```python
from build123d import *

# Parameters (mm, degrees)
WEB_1_DEPTH                   = 22
CRANKPIN_1_SKETCH_R           = 22.5
CRANKPIN_1_45_DEPTH           = 35
WEB_2_DEPTH                   = 25
CRANKPIN_2_SKETCH_R           = 22.5
CRANKPIN_2_45_DEPTH           = 35
WEB_3_DEPTH                   = 22
CENTRE_MAIN_JOURNAL_SKETCH_R  = 25
CENTRE_MAIN_JOURNAL_50_DEPTH  = 45
WEB_4_DEPTH                   = 22
CRANKPIN_3_SKETCH_R           = 22.5
CRANKPIN_3_45_DEPTH           = 35
WEB_5_DEPTH                   = 25
CRANKPIN_4_SKETCH_R           = 22.5
CRANKPIN_4_45_DEPTH           = 35
WEB_6_DEPTH                   = 22
FRONT_START                   = 45
FRONT_JOURNAL_SKETCH_R        = 22.5
FRONT_JOURNAL_45_DEPTH        = 45
FRONT_SHAFT_SKETCH_R          = 25
FRONT_SHAFT_50_DEPTH          = 100
NOSE_SKETCH_R                 = 12.5
NOSE_25_DEPTH                 = 20
FLANGE_BOLT_HOLES_SKETCH_R    = 6
FLANGE_BOLT_HOLES_4X_12_DEPTH = 20
KEYWAY_SKETCH_W               = 5
KEYWAY_SKETCH_H               = 10
KEYWAY_10X5_DEPTH             = 110


with BuildPart() as part:
    # Flange Profile Sketch → Flange and Rear Shaft (revolve)
    with BuildSketch(Plane.XY, mode=Mode.PRIVATE) as flange_and_rear_shaft_sk:
        Polygon((0, 0), (0, 60), (16, 60), (16, 22.5), (78, 22.5), (78, 0), align=None)
    revolve(flange_and_rear_shaft_sk.sketch.rotate(Axis((-89.086419753, 0, 0), (1, 0, 0)), 90), axis=Axis((-89.086419753, 0, 0), (1, 0, 0)))

    # Web 1 Sketch → Web 1 (add)
    with BuildSketch(Plane(origin=(78, 0, 0), x_dir=(0, 0, -1), z_dir=(1, 0, 0))):
        with BuildLine():
            Line((0, -27.5), (-40, -27.5))
            ThreePointArc((-40, -27.5), (-67.5, 0), (-40, 27.5))
            Line((-40, 27.5), (0, 27.5))
            ThreePointArc((0, 27.5), (27.5, 0), (0, -27.5))
        make_face()
    extrude(amount=WEB_1_DEPTH)

    # Crankpin 1 Sketch → Crankpin 1 Ø45 (add)
    with BuildSketch(Plane(origin=(100, 0, 0), x_dir=(0, 0, -1), z_dir=(1, 0, 0))):
        with Locations((-40, 0)):
            Circle(CRANKPIN_1_SKETCH_R)
    extrude(amount=CRANKPIN_1_45_DEPTH)

    # Web 2 Sketch → Web 2 (add)
    with BuildSketch(Plane(origin=(135, 0, 0), x_dir=(0, 0, -1), z_dir=(1, 0, 0))):
        with BuildLine():
            Line((-40, 27.5), (40, 27.5))
            ThreePointArc((40, 27.5), (67.5, 0), (40, -27.5))
            Line((40, -27.5), (-40, -27.5))
            ThreePointArc((-40, -27.5), (-67.5, 0), (-40, 27.5))
        make_face()
    extrude(amount=WEB_2_DEPTH)

    # Crankpin 2 Sketch → Crankpin 2 Ø45 (add)
    with BuildSketch(Plane(origin=(160, 0, 0), x_dir=(0, 0, -1), z_dir=(1, 0, 0))):
        with Locations((40, 0)):
            Circle(CRANKPIN_2_SKETCH_R)
    extrude(amount=CRANKPIN_2_45_DEPTH)

    # Web 3 Sketch → Web 3 (add)
    with BuildSketch(Plane(origin=(195, 0, 0), x_dir=(0, 0, -1), z_dir=(1, 0, 0))):
        with BuildLine():
            Line((40, -27.5), (0, -27.5))
            ThreePointArc((0, -27.5), (-27.5, 0), (0, 27.5))
            Line((0, 27.5), (40, 27.5))
            ThreePointArc((40, 27.5), (67.5, 0), (40, -27.5))
        make_face()
    extrude(amount=WEB_3_DEPTH)

    # Centre Main Journal Sketch → Centre Main Journal Ø50 (add)
    with BuildSketch(Plane(origin=(217, 0, 0), x_dir=(0, 0, -1), z_dir=(1, 0, 0))):
        with Locations(Location((0, 0, 0), (0, 0, 180))):
            Circle(CENTRE_MAIN_JOURNAL_SKETCH_R)
    extrude(amount=CENTRE_MAIN_JOURNAL_50_DEPTH)

    # Web 4 Sketch → Web 4 (add)
    with BuildSketch(Plane(origin=(262, 0, 0), x_dir=(0, 0, -1), z_dir=(1, 0, 0))):
        with BuildLine():
            Line((0, 27.5), (40, 27.5))
            ThreePointArc((40, 27.5), (67.5, 0), (40, -27.5))
            Line((40, -27.5), (0, -27.5))
            ThreePointArc((0, -27.5), (-27.5, 0), (0, 27.5))
        make_face()
    extrude(amount=WEB_4_DEPTH)

    # Crankpin 3 Sketch → Crankpin 3 Ø45 (add)
    with BuildSketch(Plane(origin=(284, 0, 0), x_dir=(0, 0, -1), z_dir=(1, 0, 0))):
        with Locations((40, 0)):
            Circle(CRANKPIN_3_SKETCH_R)
    extrude(amount=CRANKPIN_3_45_DEPTH)

    # Web 5 Sketch → Web 5 (add)
    with BuildSketch(Plane(origin=(319, 0, 0), x_dir=(0, 0, -1), z_dir=(1, 0, 0))):
        with BuildLine():
            Line((40, -27.5), (-40, -27.5))
            ThreePointArc((-40, -27.5), (-67.5, 0), (-40, 27.5))
            Line((-40, 27.5), (40, 27.5))
            ThreePointArc((40, 27.5), (67.5, 0), (40, -27.5))
        make_face()
    extrude(amount=WEB_5_DEPTH)

    # Crankpin 4 Sketch → Crankpin 4 Ø45 (add)
    with BuildSketch(Plane(origin=(344, 0, 0), x_dir=(0, 0, -1), z_dir=(1, 0, 0))):
        with Locations((-40, 0)):
            Circle(CRANKPIN_4_SKETCH_R)
    extrude(amount=CRANKPIN_4_45_DEPTH)

    # Web 6 Sketch → Web 6 (add)
    with BuildSketch(Plane(origin=(379, 0, 0), x_dir=(0, 0, -1), z_dir=(1, 0, 0))):
        with BuildLine():
            Line((-40, 27.5), (0, 27.5))
            ThreePointArc((0, 27.5), (27.5, 0), (0, -27.5))
            Line((0, -27.5), (-40, -27.5))
            ThreePointArc((-40, -27.5), (-67.5, 0), (-40, 27.5))
        make_face()
    extrude(amount=WEB_6_DEPTH)

    # Front Journal Sketch → Front Journal Ø45 (add)
    with BuildSketch(Plane(origin=(401, 0, 0), x_dir=(0, 0, -1), z_dir=(1, 0, 0)).offset(FRONT_START)):
        with Locations(Location((0, 0, 0), (0, 0, 180))):
            Circle(FRONT_JOURNAL_SKETCH_R)
    extrude(amount=-FRONT_JOURNAL_45_DEPTH)

    # Front Shaft Sketch → Front Shaft Ø50 (add)
    with BuildSketch(Plane(origin=(446, 0, 0), x_dir=(0, 0, -1), z_dir=(1, 0, 0))):
        with Locations(Location((0, 0, 0), (0, 0, 180))):
            Circle(FRONT_SHAFT_SKETCH_R)
    extrude(amount=FRONT_SHAFT_50_DEPTH)

    # Nose Sketch → Nose Ø25 (add)
    with BuildSketch(Plane(origin=(546, 0, 0), x_dir=(0, 0, -1), z_dir=(1, 0, 0))):
        Circle(NOSE_SKETCH_R)
    extrude(amount=NOSE_25_DEPTH)

    # Flange Bolt Holes Sketch → Flange Bolt Holes 4xØ12 (cut)
    with BuildSketch(Plane.ZY):
        with Locations((0, 40)):
            Circle(FLANGE_BOLT_HOLES_SKETCH_R)
        with Locations((40, 0)):
            Circle(FLANGE_BOLT_HOLES_SKETCH_R)
        with Locations((0, -40)):
            Circle(FLANGE_BOLT_HOLES_SKETCH_R)
        with Locations((-40, 0)):
            Circle(FLANGE_BOLT_HOLES_SKETCH_R)
    extrude(amount=-FLANGE_BOLT_HOLES_4X_12_DEPTH, mode=Mode.SUBTRACT)

    # Keyway Sketch → Keyway 10x5 (cut)
    with BuildSketch(Plane(origin=(546, 0, 0), x_dir=(0, 0, -1), z_dir=(1, 0, 0))):
        with Locations((-25, 0)):
            Rectangle(KEYWAY_SKETCH_W, KEYWAY_SKETCH_H)
    extrude(amount=-KEYWAY_10X5_DEPTH, mode=Mode.SUBTRACT)


solid = part.part
```
Geometry: final body of the model. Coordinates: model frame, mm. A direction names the side the tool comes from. Coordinates: 2 decimals unless noted, no trailing zeros. Order: outer loops, then holes, each group sorted by start corner. A loop starts at its lowest first (then second) coordinate and runs counter-clockwise, first axis right, second up. Notation, with made-up numbers: (67, 8) -> (120, 8) arc R20 cw to (120, 27) -> close; hole circle Ø8 at (22.25, -9). An arc over 180 degrees is marked (long way). Use CSV: the item, a comma, the result in double quotes.
1) Access query for faces 1 (the cylindrical face through (389.846, -0.605, 67.493)), 2 (the cylindrical face through (47.434, 19.961, 10.382)), 3 (the flat face through (147, 27.5, 1)), 4 (the flat face through (273, -27.5, -20)), 5 (the cylindrical face through (205.846, 0.605, -67.493)). Directions: +Z, -Z, +X, -X, +Y, -Y. A direction counts if a zero-diameter tool reaches every point of the face in a straight line with its end or side. Return the directions, or none.
Findings:
face 1,"+Z, +X"
face 2,"none"
face 3,"+Z, -Z, +X, +Y"
face 4,"+Z, -Z, +X, -Y"
face 5,"-Z, +X"
2) Mould query, pull axis X, two halves, no side actions, for faces 6 (the flat face through (546, 5, -12)), 7 (the flat face through (331, 27.5, 1)), 8 (the flat face through (135, 0, -16)). Classes: +X half, -X half, draft (parallel to the pull), parting line (faces both ways), or undercut.
Findings:
face 6,"+X half"
face 7,"draft"
face 8,"undercut"
3) Pin query (flat end, axial travel): pin 1 Ø16.5 at (y, z) = (1, 32) entering from -X; pin 2 Ø10 at (x, y) = (102.5, -9) entering from +Z; pin 3 Ø5 at (x, z) = (85.5, 1) entering from -Y; pin 4 Ø1.6 at (x, z) = (490, 24) entering from -Y. Return the tip coordinate at first contact, or that it passes through.
Findings:
pin 1,"stops at x = 0"
pin 2,"stops at z = 67.1"
pin 3,"stops at y = -27.5"
pin 4,"stops at y = -9.31"
4) Section B-B on z = -52. Output: boundary loops of the cut face in (x, y).
Findings:
outline,"(0, -29.93) -> (16, -29.93) -> (16, 29.93) -> (0, 29.93) -> close; (135, -24.74) -> (160, -24.74) -> (160, -19.03) -> (195, -19.03) -> (195, -24.74) -> (217, -24.74) -> (217, 24.74) -> (195, 24.74) -> (195, 19.03) -> (160, 19.03) -> (160, 24.74) -> (135, 24.74) -> close; (262, -24.74) -> (284, -24.74) -> (284, -19.03) -> (319, -19.03) -> (319, -24.74) -> (344, -24.74) -> (344, 24.74) -> (319, 24.74) -> (319, 19.03) -> (284, 19.03) -> (284, 24.74) -> (262, 24.74) -> close"
5) Line query: line 1 (Y direction, x = 7, z = 0); line 2 (X direction, y = -4, z = 0.5); line 3 (X direction, y = -7, z = 50.5). Output: solid intervals per line, ascending.
Findings:
line 1,"y = -60 to -46, -34 to 34, 46 to 60"
line 2,"x = 0 to 100, 135 to 160, 195 to 284, 319 to 344, 379 to 566"
line 3,"x = 0 to 16, 78 to 160, 319 to 401"
6) Section C-C on x = 392.5. Output: boundary loops of the cut face in (y, z), then the cut area to 3 significant figures.
Findings:
outline,"(-27.5, 0) arc R27.5 ccw to (27.5, 0) -> (27.5, 40) arc R27.5 ccw to (-27.5, 40) -> close"
area,"4,580 mm^2"
7) Section A-A on y = 40. Output: boundary loops of the cut face in (x, z).
Findings:
outline,"(0, -44.72) -> (16, -44.72) -> (16, -6) -> (0, -6) -> close; (0, 6) -> (16, 6) -> (16, 44.72) -> (0, 44.72) -> close"
